Part model, mm, in its own coordinate system. A direction names the side the tool comes from. Give positions to 0.01 mm unless a question says otherwise; leave off trailing zeros. Write each loop counter-clockwise with the first axis right and the second up, starting at its lowest first coordinate (ties: lowest second). Pieces come first, ordered by that corner, then holes.
```python
from build123d import *

# Parameters (mm, degrees)
CUT_EXTRUDE1_REACH = 123.809
SKETCH2_R          = 6.25
SKETCH2_W          = 90
SKETCH2_H          = 12
FILLET1_R          = 10


with BuildPart() as part:
    # Sketch1 → Revolve-Thin2 (revolve)
    with BuildSketch(Plane(origin=(0, 0, 0), x_dir=(0, 0, -1), z_dir=(1, 0, 0)), mode=Mode.PRIVATE) as revolve_thin2_sk:
        with BuildLine():
            Line((0, 49.8), (-30.4, 49.8))
            ThreePointArc((-30.4, 49.8), (-33.652691193, 51.147308807), (-35, 54.4))
            Line((-35, 54.4), (-35, 82.5))
            Line((-35, 82.5), (-33.4, 82.5))
            Line((-33.4, 82.5), (-33.4, 54.4))
            ThreePointArc((-33.4, 54.4), (-32.521320344, 52.278679656), (-30.4, 51.4))
            Line((-30.4, 51.4), (0, 51.4))
            Line((0, 51.4), (0, 49.8))
        make_face()
    revolve(revolve_thin2_sk.sketch.rotate(Axis((0, 0, 0), (0, 0, 1)), 90), axis=Axis((0, 0, 0), (0, 0, 1)))

    # Sketch2 → Cut-Extrude1 (cut, up to next)
    with BuildSketch(Plane.XY.offset(35), mode=Mode.PRIVATE) as cut_extrude1_sk1:
        with Locations((-60.4567221, 40.015431435)):
            Circle(SKETCH2_R)
    cut_extrude1_tool1 = extrude(cut_extrude1_sk1.sketch, amount=-CUT_EXTRUDE1_REACH, mode=Mode.PRIVATE) & part.part
    # Sketch2 → Cut-Extrude1 (cut, up to next)
    with BuildSketch(Plane.XY.offset(35), mode=Mode.PRIVATE) as cut_extrude1_sk2:
        with Locations((36.25, 62.786841774)):
            Circle(SKETCH2_R)
    cut_extrude1_tool2 = extrude(cut_extrude1_sk2.sketch, amount=-CUT_EXTRUDE1_REACH, mode=Mode.PRIVATE) & part.part
    # Sketch2 → Cut-Extrude1 (cut, up to next)
    with BuildSketch(Plane.XY.offset(35), mode=Mode.PRIVATE) as cut_extrude1_sk3:
        with Locations((67.455273679, 26.571338938)):
            Circle(SKETCH2_R)
    cut_extrude1_tool3 = extrude(cut_extrude1_sk3.sketch, amount=-CUT_EXTRUDE1_REACH, mode=Mode.PRIVATE) & part.part
    # Sketch2 → Cut-Extrude1 (cut, up to next)
    with BuildSketch(Plane.XY.offset(35), mode=Mode.PRIVATE) as cut_extrude1_sk4:
        with Locations((51.265241636, -51.265241636)):
            Circle(SKETCH2_R)
    cut_extrude1_tool4 = extrude(cut_extrude1_sk4.sketch, amount=-CUT_EXTRUDE1_REACH, mode=Mode.PRIVATE) & part.part
    # Sketch2 → Cut-Extrude1 (cut, up to next)
    with BuildSketch(Plane.XY.offset(35), mode=Mode.PRIVATE) as cut_extrude1_sk5:
        with Locations((-16.92478888, -70.496819229)):
            Circle(SKETCH2_R)
    cut_extrude1_tool5 = extrude(cut_extrude1_sk5.sketch, amount=-CUT_EXTRUDE1_REACH, mode=Mode.PRIVATE) & part.part
    # Sketch2 → Cut-Extrude1 (cut, up to next)
    with BuildSketch(Plane.XY.offset(35), mode=Mode.PRIVATE) as cut_extrude1_sk6:
        with Locations((-71.398562093, 12.589492881)):
            Circle(SKETCH2_R)
    cut_extrude1_tool6 = extrude(cut_extrude1_sk6.sketch, amount=-CUT_EXTRUDE1_REACH, mode=Mode.PRIVATE) & part.part
    # Sketch2 → Cut-Extrude1 (cut, up to next)
    with BuildSketch(Plane.XY.offset(35), mode=Mode.PRIVATE) as cut_extrude1_sk7:
        with Locations((0, 78.5)):
            Rectangle(SKETCH2_W, SKETCH2_H)
    cut_extrude1_tool7 = extrude(cut_extrude1_sk7.sketch, amount=-CUT_EXTRUDE1_REACH, mode=Mode.PRIVATE) & part.part
    add(cut_extrude1_tool1.solids().sort_by_distance((-60.456722, 40.015431, 35))[0], mode=Mode.SUBTRACT)
    add(cut_extrude1_tool2.solids().sort_by_distance((36.25, 62.786842, 35))[0], mode=Mode.SUBTRACT)
    add(cut_extrude1_tool3.solids().sort_by_distance((67.455274, 26.571339, 35))[0], mode=Mode.SUBTRACT)
    add(cut_extrude1_tool4.solids().sort_by_distance((51.265242, -51.265242, 35))[0], mode=Mode.SUBTRACT)
    add(cut_extrude1_tool5.solids().sort_by_distance((-16.924789, -70.496819, 35))[0], mode=Mode.SUBTRACT)
    add(cut_extrude1_tool6.solids().sort_by_distance((-71.398562, 12.589493, 35))[0], mode=Mode.SUBTRACT)
    add(cut_extrude1_tool7.solids().sort_by_distance((0, 78.5, 35))[0], mode=Mode.SUBTRACT)

    # Fillet1
    fillet1_edges = [part.edges().sort_by_distance(p)[0] for p in [
        (-39.37003937, 72.5, 34.2),
        (39.37003937, 72.5, 34.2),
    ]]
    fillet(fillet1_edges, radius=FILLET1_R)


solid = part.part
```
1) Saw through at B-B, the plane y = 0. Write the cut outline in (x, z), then the cut area to 3 significant figures.
Answers follow:
outline: (-82.5, 33.4) - (-54.4, 33.4) arc R3 cw to (-51.4, 30.4) - (-51.4, 0) - (-49.8, 0) - (-49.8, 30.4) arc R4.6 ccw to (-54.4, 35) - (-82.5, 35) - close; (49.8, 0) - (51.4, 0) - (51.4, 30.4) arc R3 cw to (54.4, 33.4) - (82.5, 33.4) - (82.5, 35) - (54.4, 35) arc R4.6 ccw to (49.8, 30.4) - close
area: 206 mm2
2) 3-axis set-ups, long thin cutter, end or side, ignore diameter. For faces 4 (the face through (38, -41, 33.4)), 5 (the face through (-77.643, 12.864, 34.211)): which of +Z, -Z, +X, -X, +Y, -Y reach the whole face in a straight line?
Answers follow:
face 4: -Z
face 5: +Z, -Z
3) Wall check: L1, parallel to X at y = -1, z = 10; L2, parallel to Z at x = -54, y = -28.5; L3, parallel to X at y = 45, z = 17.5. Give the ranges that are in metal, low to high.
Answers follow:
L1: x = -51.39 to -49.79, 49.79 to 51.39
L2: z = 33.4 to 35
L3: x = -24.84 to -21.33, 21.33 to 24.84
4) Saw through at A-A, the plane x = 0. Write the cut outline in (y, z), then the cut area to 3 significant figures.
Answers follow:
outline: (-82.5, 33.4) - (-54.4, 33.4) arc R3 cw to (-51.4, 30.4) - (-51.4, 0) - (-49.8, 0) - (-49.8, 30.4) arc R4.6 ccw to (-54.4, 35) - (-82.5, 35) - close; (49.8, 0) - (51.4, 0) - (51.4, 30.4) arc R3 cw to (54.4, 33.4) - (72.5, 33.4) - (72.5, 35) - (54.4, 35) arc R4.6 ccw to (49.8, 30.4) - close
area: 190 mm2
5) Saw through at C-C, the plane z = 15.5. Write the cut outline in (x, y).
Answers follow:
outline: circle Ø102.8 at (0, 0); hole circle Ø99.6 at (0, 0)
6) Saw through at D-D, the plane y = 59. Write the cut outline in (x, z), then the cut area to 3 significant figures.
Answers follow:
outline: (-57.66, 33.4) - (31.28, 33.4) - (31.28, 35) - (-57.66, 35) - close; (41.22, 33.4) - (57.66, 33.4) - (57.66, 35) - (41.22, 35) - close
area: 169 mm2
7) Pin check, flat tips, straight feed: pin 1 Ø14.5 at (x, y) = (36.25, 62.79) entering from -Z; pin 2 Ø5 at (y, z) = (-28.5, 14) entering from +X; pin 3 Ø7.5 at (x, y) = (51.27, -51.27) entering from -Z; pin 4 Ø6 at (y, z) = (12.5, 22.5) entering from +X. Stop position of each tip, or through.
Answers follow:
pin 1: stops at z = 33.4
pin 2: stops at x = 44.34
pin 3: passes through
pin 4: stops at x = 50.51
8) Two-plate mould, pull along X, no slides. Class faces 1 (the face through (39.52, 30.3, 15.41)), 2 (the face through (-38, -41, 35)), 3 (the face through (-3.014, -82.445, 34.189)): +X half, -X half, draft (parallel to the pull), parting line (faces both ways), or undercut.
Answers follow:
face 1: undercut
face 2: draft
face 3: parting line
